Geometry check sheet. Reference: the model listing, model coordinates, mm. A direction names the side the tool comes from. Coordinates: 2 decimals unless noted, no trailing zeros. Write each loop counter-clockwise with the first axis right and the second up, starting at its lowest first coordinate (ties: lowest second). Pieces come first, ordered by that corner, then holes. Notation, with made-up numbers: M 67.5,69.25 L 101.5,69.25 A15 cw 101.5,81.25 Z; hole C 41.25,18.25 d4. An arc over 180 degrees is marked long. Put each result on its own line as item: value. Start each with the question number.
1) Cross-section at C-C on y = 4. Record the cut outline in (x, z).
2) Set-up check for faces 4 (the flat face through (13, 0, 1)), 5 (the flat face through (0.2, 13.5, 77.3)): record each of +Z, -Z, +X, -X, +Y, -Y from which the full face is reachable in a straight line by a thin tool's end or side.
3) Cross-section at D-D on z = -76.5. Record the cut outline in (x, y), plus the area to 3 significant figures.
4) Mould release check, pull along Y, two halves, no side actions. Record for faces 1 (the flat face through (-0.2, 13.5, -77.7)), 2 (the flat face through (0, 15, 1)), 3 (the flat face through (0, 13, 1)): released by +Y, released by -Y, zero draft, split by the parting line, or undercut.
5) Cross-section at A-A on x = -1.5. Record the cut outline in (y, z).
6) Gauge pin test, flat end, axial feed: pin 1 (12 mm diameter, centred on x = 1.5, y = -6, fed in from -Z). Record the tip position at first contact, or that the pin passes through.
7) Scan lines: line 1 along Y through (x, z) = (-2.5, 60.5); line 2 along X through (y, z) = (-10, 69.5). Record each from-to range of solid material in increasing order.
8) Cross-section at B-B on z = 55.5. Record the cut outline in (x, y).
from build123d import *

# Parameters (mm, degrees)
SKETCH_1_W          = 30
SKETCH_1_H          = 30
SKETCH_1_W_2        = 26
SKETCH_1_H_2        = 26
EXTRUDE_1_DEPTH     = 92.5
CUT_EXTRUDE_1_DEPTH = 87


with BuildPart() as part:
    # 草图1 → 凸台-拉伸1 (new, symmetric)
    with BuildSketch(Plane.XY):
        Rectangle(SKETCH_1_W, SKETCH_1_H)
        Rectangle(SKETCH_1_W_2, SKETCH_1_H_2, mode=Mode.SUBTRACT)
    extrude(amount=EXTRUDE_1_DEPTH, both=True)

    # 草图2 → 切除-拉伸1 (cut)
    with BuildSketch(Plane(origin=(0, 15, 0), x_dir=(1, 0, 0), z_dir=(0, 1, 0))):
        Polygon((15, -62.5), (-15, -92.5), (15, -92.5), align=None)
        Polygon((15, 92.5), (-15, 92.5), (15, 62.5), align=None)
    extrude(amount=-CUT_EXTRUDE_1_DEPTH, mode=Mode.SUBTRACT)


solid = part.part
Answer key:
1. outline: M -15,-92.5 L -13,-90.5 L -13,90.5 L -15,92.5 Z; M 13,-64.5 L 15,-62.5 L 15,62.5 L 13,64.5 Z
2. face 4: +Z, -Z
2. face 5: +Z, +X, +Y, -Y
3. outline: M -15,-15 L 1,-15 L 1,-13 L -13,-13 L -13,13 L 1,13 L 1,15 L -15,15 Z
3. area: 116 mm²
4. face 1: zero draft
4. face 2: released by +Y
4. face 3: undercut
5. outline: M -15,-79 L -13,-79 L -13,79 L -15,79 Z; M 13,-79 L 15,-79 L 15,79 L 13,79 Z
6. pin 1: passes through
7. line 1: y = -15 to -13, 13 to 15
7. line 2: x = -15 to -13
8. outline: M -15,-15 L 15,-15 L 15,15 L -15,15 Z; hole M -13,-13 L 13,-13 L 13,13 L -13,13 Z
